The figure shows three views and two pictorial views of one solid part (mm, origin at its lowest corner). Answer the questions. Coordinates: 2 decimals unless noted, no trailing zeros. Order: outer loops, then holes, each group sorted by start corner. A loop starts at its lowest first (then second) coordinate and runs counter-clockwise, first axis right, second up. Notation, with made-up numbers: (33, -17) -> (44, -17) arc R20 ccw to (44, 17) -> close; hole circle Ø11 at (73, 71). An arc over 180 degrees is marked (long way). Return JSON: item names as keys, results as strings. Group by question number.
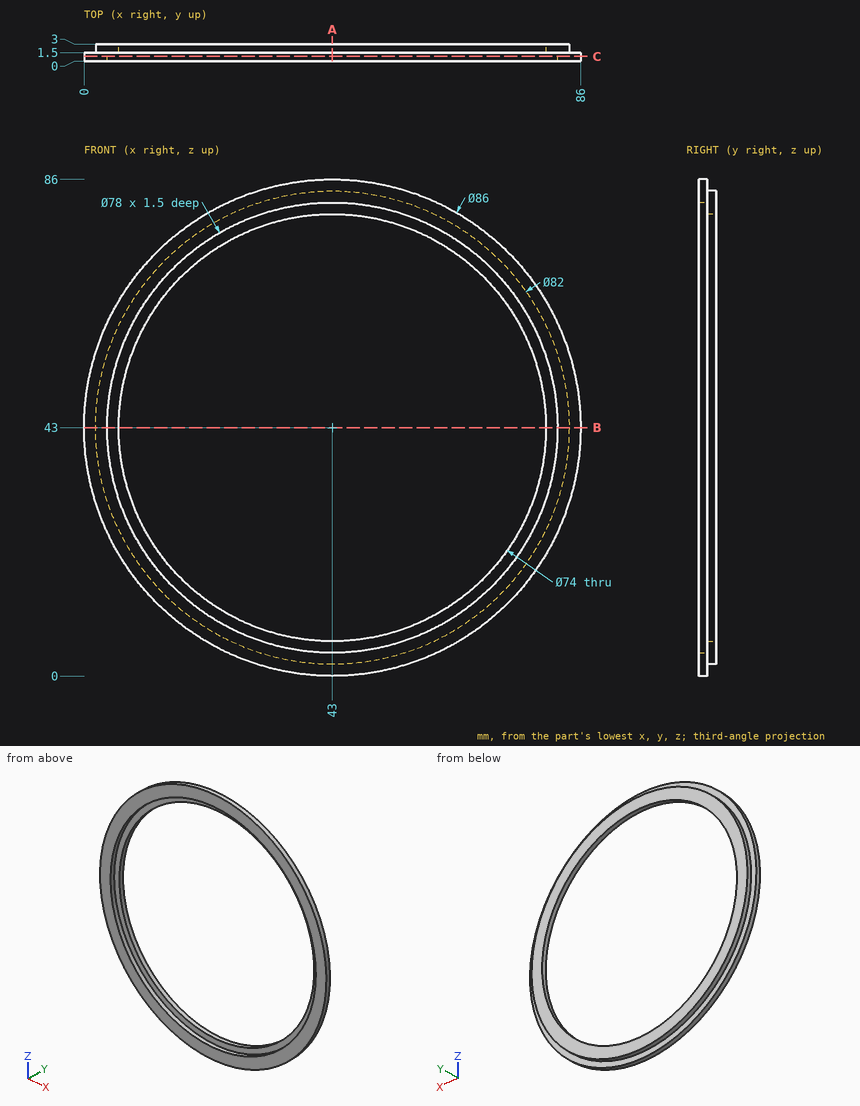
1. Find section C-C on y = 0.85. Determine the outline of the cut face in (x, z).
2. Find section A-A on x = 43. Determine the outline of the cut face in (y, z), and give its area (3 significant figures).
3. Find section B-B on z = 43. Determine the outline of the cut face in (x, y), and give its area (3 significant figures).
4. Straight lines are drawn through the part: L1, parallel to Z at x = 44, y = 2.75; L2, parallel to X at y = 0.55, z = 43; L3, parallel to X at y = 2.7, z = 11.5. For each, find the intervals that lie inside material, in ascending order.
5. Given pin 1 (23.5 mm diameter, centred on x = 62.5, z = 58, fed in from -Y); pin 2 (1 mm diameter, centred on y = 1.5, z = 24, fed in from -X); pin 3 (1 mm diameter, centred on x = 52.5, y = 1, fed in from +Z), each flat-ended and moving along its own axis, determine where each tip first touches the part or whether it passes through.
Result:
{
 "1": {"outline": "circle Ø86 at (43, 43); hole circle Ø78 at (43, 43)"},
 "2": {"outline": "(0, 0) -> (1.5, 0) -> (1.5, 2) -> (3, 2) -> (3, 6) -> (1.5, 6) -> (1.5, 4) -> (0, 4) -> close; (0, 82) -> (1.5, 82) -> (1.5, 80) -> (3, 80) -> (3, 84) -> (1.5, 84) -> (1.5, 86) -> (0, 86) -> close", "area": "24.0 mm^2"},
 "3": {"outline": "(0, 0) -> (4, 0) -> (4, 1.5) -> (6, 1.5) -> (6, 3) -> (2, 3) -> (2, 1.5) -> (0, 1.5) -> close; (80, 1.5) -> (82, 1.5) -> (82, 0) -> (86, 0) -> (86, 1.5) -> (84, 1.5) -> (84, 3) -> (80, 3) -> close", "area": "24.0 mm^2"},
 "4": {"L1": "2.01 to 6.01, 79.99 to 83.99", "L2": "0 to 4, 82 to 86", "L3": "16.76 to 23.59, 62.41 to 69.24"},
 "5": {"pin 1": "through", "pin 2": "x = 4.18", "pin 3": "z = 85.05"}
}
